Check sheet for the modelled part. Datum: model origin and axes. Units: mm. A direction names the side the tool comes from. Round coordinates to 2 decimals unless told otherwise and drop trailing zeros. Loops run counter-clockwise (first coordinate to the right, second up) from the corner with the lowest first, then second, coordinate; pieces in that order, holes last. Notation, with made-up numbers: (25.25, 78.25) -> (47.25, 78.25) arc R15 ccw to (47.25, 96.25) -> close; hole circle Ø7 at (28.5, 67.25). An arc over 180 degrees is marked (long way). Return JSON: item names as keys, results as strings.
from build123d import *

# Parameters (mm, degrees)
SKETCH1_R           = 17
BOSS_EXTRUDE1_DEPTH = 4
CUT_EXTRUDE1_DEPTH  = 2
SKETCH3_R           = 2
SKETCH3_R_2         = 1.5
CUT_EXTRUDE2_DEPTH  = 4
FILLET1_R           = 1


with BuildPart() as part:
    # Sketch1 → Boss-Extrude1 (new body)
    with BuildSketch(Plane.XY):
        Circle(SKETCH1_R)
    extrude(amount=BOSS_EXTRUDE1_DEPTH)

    # Sketch2 → Cut-Extrude1 (cut)
    with BuildSketch(Plane.XY.offset(4)):
        with BuildLine():
            Line((2.5, 4.5), (2.5, -4.5))
            ThreePointArc((2.5, -4.5), (0, -7), (-2.5, -4.5))
            Line((-2.5, -4.5), (-2.5, 4.5))
            ThreePointArc((-2.5, 4.5), (0, 7), (2.5, 4.5))
        make_face()
    extrude(amount=-CUT_EXTRUDE1_DEPTH, mode=Mode.SUBTRACT)

    # Sketch3 → Cut-Extrude2 (cut)
    with BuildSketch(Plane.XY.offset(4)):
        with Locations((0, 11)):
            Circle(SKETCH3_R)
        with Locations((11, 0)):
            Circle(SKETCH3_R)
        with Locations((-7.778174593, 7.778174593)):
            Circle(SKETCH3_R_2)
        with Locations((7.778174593, -7.778174593)):
            Circle(SKETCH3_R_2)
    extrude(amount=-CUT_EXTRUDE2_DEPTH, mode=Mode.SUBTRACT)

    # Fillet1
    fillet1_edges = [part.edges().sort_by_distance(p)[0] for p in [
        (-17, 0, 4),
    ]]
    fillet(fillet1_edges, radius=FILLET1_R)


solid = part.part
Q1. Section check C-C (z = 1.55). Record the boundary of the cut face in (x, y), then the cut area to 3 significant figures.
Results list:
{"outline": "circle Ø34 at (0, 0); hole circle Ø3 at (-7.78, 7.78); hole circle Ø4 at (0, 11); hole circle Ø3 at (7.78, -7.78); hole circle Ø4 at (11, 0)", "area": "869 mm^2"}
Q2. Go/stop test with flat-tipped pins: pin 1 (1.6 mm diameter, centred on y = -2, z = 2.5, fed in from -X); pin 2 (1.5 mm diameter, centred on x = 3.5, z = 3, fed in from -Y); pin 3 (2.5 mm diameter, centred on x = -0.5, y = -1.5, fed in from +Z); pin 4 (2.5 mm diameter, centred on x = 7.78, y = -7.78, fed in from -Z). Record where each tip stops, or that it passes through.
Results list:
{"pin 1": "x = -16.96", "pin 2": "y = -16.78", "pin 3": "z = 2", "pin 4": "through"}
Q3. Material ranges on line 1 (Y direction, x = 0, z = 2.7); line 2 (X direction, y = -8, z = 2.75); line 3 (X direction, y = 8, z = 2.55), recorded low to high.
Results list:
{"line 1": "-17 to -7, 7 to 9, 13 to 17", "line 2": "-15 to 6.29, 9.26 to 15", "line 3": "-15 to -9.26, -6.29 to 15"}
Q4. Section check B-B (y = 0). Record the boundary of the cut face in (x, z), then the cut area to 3 significant figures.
Results list:
{"outline": "(-17, 0) -> (9, 0) -> (9, 4) -> (2.5, 4) -> (2.5, 2) -> (-2.5, 2) -> (-2.5, 4) -> (-16, 4) arc R1 ccw to (-17, 3) -> close; (13, 0) -> (17, 0) -> (17, 3) arc R1 ccw to (16, 4) -> (13, 4) -> close", "area": "110 mm^2"}
Q5. Section check A-A (x = 0). Record the boundary of the cut face in (y, z), then the cut area to 3 significant figures.
Results list:
{"outline": "(-17, 0) -> (9, 0) -> (9, 4) -> (7, 4) -> (7, 2) -> (-7, 2) -> (-7, 4) -> (-16, 4) arc R1 ccw to (-17, 3) -> close; (13, 0) -> (17, 0) -> (17, 3) arc R1 ccw to (16, 4) -> (13, 4) -> close", "area": "91.6 mm^2"}
Q6. Tool access check on faces 1 (the flat face through (0, 0, 2)), 2 (the cylindrical face through (-7.973, 9.265, 2.028)). Record the directions out of +Z, -Z, +X, -X, +Y, -Y that give a thin tool (end or side, any length) a straight path to the whole face; none if there is none.
Results list:
{"face 1": "+Z", "face 2": "+Z, -Z"}
Q7. Draft check along Y on faces 3 (the flat face through (0, 0, 0)), 4 (the cylindrical face through (9.139, 14.334, 1.479)), 5 (the flat face through (-2.5, 0, 3)). Enter one of: released by +Y, released by -Y, zero draft, split by the parting line, or undercut.
Results list:
{"face 3": "zero draft", "face 4": "split by the parting line", "face 5": "undercut"}
